```python
from build123d import *

# Parameters (mm, degrees)
SKETCH1_W           = 50
SKETCH1_H           = 10
BOSS_EXTRUDE1_DEPTH = 4
CUT_EXTRUDE1_DEPTH  = 52.14684741
CUT_EXTRUDE2_DEPTH  = 52.14684741
CUT_EXTRUDE3_DEPTH  = 52.14684741
CUT_EXTRUDE4_DEPTH  = 52.14684741
CUT_EXTRUDE5_DEPTH  = 52.14684741
CUT_EXTRUDE6_DEPTH  = 52.14684741
CUT_EXTRUDE7_DEPTH  = 52.14684741
CUT_EXTRUDE8_DEPTH  = 52.14684741


with BuildPart() as part:
    # Sketch1 → Boss-Extrude1 (new body)
    with BuildSketch(Plane.XY.offset(2)):
        with Locations((-25, 5)):
            Rectangle(SKETCH1_W, SKETCH1_H)
    extrude(amount=-BOSS_EXTRUDE1_DEPTH)

    # Sketch2 → Cut-Extrude1 (cut, through all)
    with BuildSketch(Plane(origin=(0, 0, -2), x_dir=(-1, 0, 0), z_dir=(0, 0, -1))):
        Polygon((40.976059531, 0), (45.573940469, 0), (43.936074414, 4.5), (42.613925586, 4.5), align=None)
    extrude(amount=-CUT_EXTRUDE1_DEPTH, mode=Mode.SUBTRACT)

    # Sketch3 → Cut-Extrude2 (cut, through all)
    with BuildSketch(Plane(origin=(0, 0, -2), x_dir=(-1, 0, 0), z_dir=(0, 0, -1))):
        Polygon((34.692059531, 0), (39.289940469, 0), (37.652074414, 4.5), (36.329925586, 4.5), align=None)
    extrude(amount=-CUT_EXTRUDE2_DEPTH, mode=Mode.SUBTRACT)

    # Sketch4 → Cut-Extrude3 (cut, through all)
    with BuildSketch(Plane(origin=(0, 0, -2), x_dir=(-1, 0, 0), z_dir=(0, 0, -1))):
        Polygon((28.408059531, 0), (33.005940469, 0), (31.368074414, 4.5), (30.045925586, 4.5), align=None)
    extrude(amount=-CUT_EXTRUDE3_DEPTH, mode=Mode.SUBTRACT)

    # Sketch5 → Cut-Extrude4 (cut, through all)
    with BuildSketch(Plane(origin=(0, 0, -2), x_dir=(-1, 0, 0), z_dir=(0, 0, -1))):
        Polygon((22.124059531, 0), (26.721940469, 0), (25.084074414, 4.5), (23.761925586, 4.5), align=None)
    extrude(amount=-CUT_EXTRUDE4_DEPTH, mode=Mode.SUBTRACT)

    # Sketch6 → Cut-Extrude5 (cut, through all)
    with BuildSketch(Plane(origin=(0, 0, -2), x_dir=(-1, 0, 0), z_dir=(0, 0, -1))):
        Polygon((15.840059531, 0), (20.437940469, 0), (18.800074414, 4.5), (17.477925586, 4.5), align=None)
    extrude(amount=-CUT_EXTRUDE5_DEPTH, mode=Mode.SUBTRACT)

    # Sketch7 → Cut-Extrude6 (cut, through all)
    with BuildSketch(Plane(origin=(0, 0, -2), x_dir=(-1, 0, 0), z_dir=(0, 0, -1))):
        Polygon((9.556059531, 0), (14.153940469, 0), (12.516074414, 4.5), (11.193925586, 4.5), align=None)
    extrude(amount=-CUT_EXTRUDE6_DEPTH, mode=Mode.SUBTRACT)

    # Sketch8 → Cut-Extrude7 (cut, through all)
    with BuildSketch(Plane(origin=(0, 0, -2), x_dir=(-1, 0, 0), z_dir=(0, 0, -1))):
        Polygon((3.272059531, 0), (7.869940469, 0), (6.232074414, 4.5), (4.909925586, 4.5), align=None)
    extrude(amount=-CUT_EXTRUDE7_DEPTH, mode=Mode.SUBTRACT)

    # Sketch9 → Cut-Extrude8 (cut, through all)
    with BuildSketch(Plane(origin=(0, 0, -2), x_dir=(-1, 0, 0), z_dir=(0, 0, -1))):
        Polygon((48.897925586, 4.5), (47.260059531, 0), (50, 0), (50, 4.5), align=None)
    extrude(amount=-CUT_EXTRUDE8_DEPTH, mode=Mode.SUBTRACT)

    # Sketch10 → Revolve1 (revolve)
    with BuildSketch(Plane.XY):
        Polygon((0, 9), (0, 5), (58, 5), (58, 13), (50, 13), (50, 9), align=None)
    revolve(axis=Axis((0, 5, 0), (1, 0, 0)))


solid = part.part
```
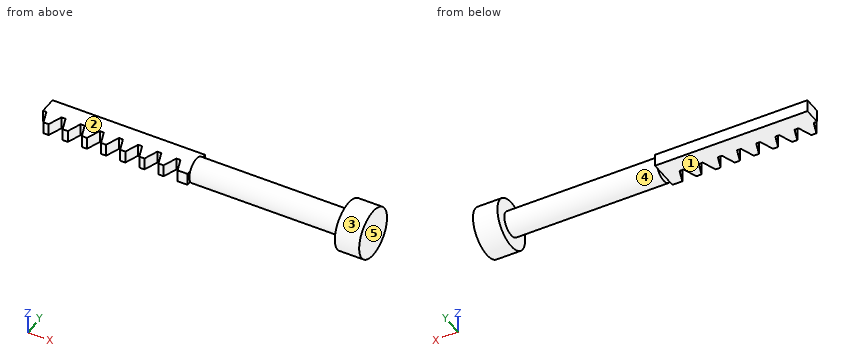
Can you work these out from the model? Positions are in its coordinate system, mm. Face numbers are marked on the shaded views. A direction names the side the tool comes from. Coordinates: 2 decimals unless noted, no trailing zeros. Write each loop counter-clockwise with the first axis right and the second up, starting at its lowest first coordinate (ties: lowest second). Pieces come first, ordered by that corner, then holes. Notation, with made-up numbers: (3.25, -2) - (17.25, -2) arc R20 ccw to (17.25, 21) - close; hole circle Ø7 at (70, 21). An arc over 180 degrees is marked (long way). Return JSON: item names as keys, results as strings.
Q1. If we section it at A-A (y = 7.5): Please give me the cut outline in (x, z), then the cut area to 3 significant figures.
Computed values:
{"outline": "(-50, -2) - (0, -2) - (0, -3.12) - (50, -3.12) - (50, -7.6) - (58, -7.6) - (58, 7.6) - (50, 7.6) - (50, 3.12) - (0, 3.12) - (0, 2) - (-50, 2) - close", "area": "634 mm2"}
Q2. Please list where these lines run through material, in increasing order: L1, parallel to X at y = 10.25, z = -4.5; L2, parallel to Z at x = -5.5, y = 9; L3, parallel to Z at x = 9, y = 5.5. Write a range as from..to.
Computed values:
{"L1": "x = 50..58", "L2": "z = -2..2", "L3": "z = -3.97..3.97"}
Q3. Thinking about a two-plate mould opening in X: for the marked faces 3, 4 and 5, which applies, +X half, -X half, draft (parallel to the pull), parting line (faces both ways), or undercut?
Computed values:
{"face 3": "draft", "face 4": "undercut", "face 5": "+X half"}
Q4. If we section it at D-D (z = -5.75): Please give me the cut outline in (x, y), then the cut area to 3 significant figures.
Computed values:
{"outline": "(50, -0.56) - (58, -0.56) - (58, 10.56) - (50, 10.56) - close", "area": "89.0 mm2"}
Q5. If we section it at C-C (y = 2.5): Count the separate pieces of the cut face and the enclosed holes in it, then the cut area to 3 significant figures.
Computed values:
{"separate pieces": "8", "enclosed holes": "0", "area": "549 mm2"}
Q6. If we section it at B-B (x = 21.5): Please give me the cut outline in (y, z), then the cut area to 3 significant figures.
Computed values:
{"outline": "circle Ø8 at (5, 0)", "area": "50.3 mm2"}
Q7. On a 3-axis mill with a long thin cutter (end or side, diameter ignored), from which of +Z, -Z, +X, -X, +Y, -Y can I reach the whole of each face in a straight line? I mean the marked faces 1 and 2. Say none if no direction works.
Computed values:
{"face 1": "-Z, -X, +Y, -Y", "face 2": "+Z, -X, +Y, -Y"}
Q8. I'm going to push flat-ended pins straight in: pin 1 Ø1.2 at (x, z) = (-35.5, 0) entering from +Y; pin 2 Ø1.9 at (x, z) = (-9, -0.5) entering from -Y; pin 3 Ø1.6 at (y, z) = (6, 3) entering from -X. Where does each tip first touch, or does it pass through?
Computed values:
{"pin 1": "stops at y = 10", "pin 2": "stops at y = 0", "pin 3": "stops at x = 0"}
